```python
from build123d import *

# Parameters (mm, degrees)
SKETCH_1_R      = 2.1
SKETCH_1_R_2    = 1.6
EXTRUDE_1_DEPTH = 3
CHAMFER_1_SIZE  = 13
CHAMFER_2_SIZE  = 2
FILLET_1_R      = 3


with BuildPart() as part:
    # 草图1 → 凸台-拉伸1 (new body)
    with BuildSketch(Plane(origin=(0, 0, 0), x_dir=(1, 0, 0), z_dir=(0, 1, 0))):
        Polygon((-55, -25), (-55, 25), (-39.5, 25), (-39.5, 34), (39.5, 34), (39.5, 25), (55, 25), (55, -25), (42, -25), (33.5, -8), (33.5, 28), (0, 28), (-33.5, 28), (-33.5, -8), (-42, -25), align=None)
        with Locations(Location((-47.5, 21, 0), (0, 0, 270))):
            Circle(SKETCH_1_R, mode=Mode.SUBTRACT)
        with Locations(Location((-47.5, -21, 0), (0, 0, 270))):
            Circle(SKETCH_1_R, mode=Mode.SUBTRACT)
        with Locations(Location((47.5, -21, 0), (0, 0, 270))):
            Circle(SKETCH_1_R, mode=Mode.SUBTRACT)
        with Locations(Location((47.5, 21, 0), (0, 0, 270))):
            Circle(SKETCH_1_R, mode=Mode.SUBTRACT)
        with Locations(Location((-36.5, 31, 0), (0, 0, 270))):
            Circle(SKETCH_1_R_2, mode=Mode.SUBTRACT)
        with Locations(Location((-36.5, -5, 0), (0, 0, 270))):
            Circle(SKETCH_1_R_2, mode=Mode.SUBTRACT)
        with Locations(Location((36.5, -5, 0), (0, 0, 270))):
            Circle(SKETCH_1_R_2, mode=Mode.SUBTRACT)
        with Locations(Location((36.5, 31, 0), (0, 0, 270))):
            Circle(SKETCH_1_R_2, mode=Mode.SUBTRACT)
        with Locations(Location((-23.5, 31, 0), (0, 0, 270))):
            Circle(SKETCH_1_R_2, mode=Mode.SUBTRACT)
        with Locations(Location((23.5, 31, 0), (0, 0, 270))):
            Circle(SKETCH_1_R_2, mode=Mode.SUBTRACT)
    extrude(amount=EXTRUDE_1_DEPTH)

    # 倒角1
    chamfer_1_edges = [part.edges().sort_by_distance(p)[0] for p in [
        (33.5, 1.5, -28),
        (-33.5, 1.5, -28),
    ]]
    chamfer(chamfer_1_edges, length=CHAMFER_1_SIZE)

    # 倒角2
    chamfer_2_edges = [part.edges().sort_by_distance(p)[0] for p in [
        (55, 1.5, -25),
        (-55, 1.5, -25),
        (-39.5, 1.5, -25),
        (39.5, 1.5, -25),
    ]]
    chamfer(chamfer_2_edges, length=CHAMFER_2_SIZE)

    # 圆角1
    fillet_1_edges = [part.edges().sort_by_distance(p)[0] for p in [
        (41.5, 1.5, -25),
        (53, 1.5, -25),
        (55, 1.5, -23),
        (39.5, 1.5, -27),
        (-55, 1.5, -23),
        (-41.5, 1.5, -25),
        (-53, 1.5, -25),
        (-39.5, 1.5, -27),
        (55, 1.5, 25),
        (42, 1.5, 25),
        (33.5, 1.5, 8),
        (-33.5, 1.5, 8),
        (-42, 1.5, 25),
        (-55, 1.5, 25),
        (-39.5, 1.5, -34),
        (39.5, 1.5, -34),
        (33.5, 1.5, -15),
        (-20.5, 1.5, -28),
        (20.5, 1.5, -28),
        (-33.5, 1.5, -15),
    ]]
    fillet(fillet_1_edges, radius=FILLET_1_R)


solid = part.part
```
Could you check a few things on this model? Use its own coordinates, in mm. A direction names the side the tool comes from. Round coordinates to 2 decimals unless told otherwise and drop trailing zeros. Loops run counter-clockwise (first coordinate to the right, second up) from the corner with the lowest first, then second, coordinate; pieces in that order, holes last. Notation, with made-up numbers: (-39, 45) -> (-32, 45) arc R30 ccw to (-32, 84) -> close; hole circle Ø2 at (-18.5, 6). An arc over 180 degrees is marked (long way). Put each result on its own line as item: value.
Q1. I want a section at A-A on z = -3.5. Write out the boundary of the cut face in (x, y), and give its area (3 significant figures).
Checks:
outline: (-55, 0) -> (-33.5, 0) -> (-33.5, 3) -> (-55, 3) -> close; (33.5, 0) -> (55, 0) -> (55, 3) -> (33.5, 3) -> close
area: 129 mm2
Q2. For pin 1 Ø1.5 at (x, y) = (46, 1.5) entering from -Z; pin 2 Ø1.5 at (x, y) = (7.5, 1) entering from +Z; pin 3 Ø0.8 at (y, z) = (2, -30) entering from +X; pin 4 Ø2.5 at (x, z) = (-36.5, 5) entering from -Y, each with a flat end and sliding along its axis, tell me the tip position at first contact or that it passes through.
Checks:
pin 1: z = -25
pin 2: z = -28
pin 3: x = 39.5
pin 4: through
Q3. I want a section at B-B on x = -23.5. Write out the boundary of the cut face in (y, z).
Checks:
outline: (0, -34) -> (3, -34) -> (3, -32.6) -> (0, -32.6) -> close; (0, -29.4) -> (3, -29.4) -> (3, -25) -> (0, -25) -> close
Q4. I want a section at C-C on z = 21. Write out the boundary of the cut face in (x, y), and give its area (3 significant figures).
Checks:
outline: (-55, 0) -> (-49.6, 0) -> (-49.6, 3) -> (-55, 3) -> close; (-45.4, 0) -> (-40, 0) -> (-40, 3) -> (-45.4, 3) -> close; (40, 0) -> (45.4, 0) -> (45.4, 3) -> (40, 3) -> close; (49.6, 0) -> (55, 0) -> (55, 3) -> (49.6, 3) -> close
area: 64.8 mm2
Q5. Which directions (+Z, -Z, +X, -X, +Y, -Y) give clear straight access to the entire face, cutting with the end or side of a thin tool? Please do faces 1 (the cylindrical face through (24.58, 1.48, -32.18)), 2 (the cylindrical face through (42.26, 1.52, 24.54)), 3 (the flat face through (-47, 1, -25)).
Checks:
face 1: +Y, -Y
face 2: +Z, +Y, -Y
face 3: -Z, -X, +Y, -Y
Q6. I want a section at D-D on x = -47.5. Write out the boundary of the cut face in (y, z).
Checks:
outline: (0, -25) -> (3, -25) -> (3, -23.1) -> (0, -23.1) -> close; (0, -18.9) -> (3, -18.9) -> (3, 18.9) -> (0, 18.9) -> close; (0, 23.1) -> (3, 23.1) -> (3, 25) -> (0, 25) -> close
Q7. Please list where these lines run through material, in increasing order: line 1 (X direction, y = 1.65, z = 5); line 2 (X direction, y = 2.25, z = -31); line 3 (X direction, y = 2.1, z = -7.5). Write a range as from..to.
Checks:
line 1: -55..-38.1, -34.9..-33.5, 33.5..34.9, 38.1..55
line 2: -39.5..-38.1, -34.9..-25.1, -21.9..21.9, 25.1..34.9, 38.1..39.5
line 3: -55..-33.5, 33.5..55
Q8. Thinking about a two-plate mould opening in Z: for faces 4 (the cylindrical face through (-42.297, 1.521, 24.564)), 5 (the flat face through (47, 1, -25)), 6 (the cylindrical face through (-37.47, 1.48, -32.27)), which applies, pulls with the +Z half, pulls with the -Z half, needs draft (parallel to the pull), parting line crosses it, or undercut?
Checks:
face 4: pulls with the +Z half
face 5: pulls with the -Z half
face 6: undercut
